Work out the finished part from the listing and answer in its coordinate system (mm). Face numbers are marked on the shaded views. Round coordinates to 2 decimals unless told otherwise and drop trailing zeros. Loops run counter-clockwise (first coordinate to the right, second up) from the corner with the lowest first, then second, coordinate; pieces in that order, holes last. Notation, with made-up numbers: M 1.5,3 L 17.5,3 A32 ccw 17.5,41 Z; hole C 18.5,32.5 d1. An arc over 180 degrees is marked long. One line per item, written item: value.
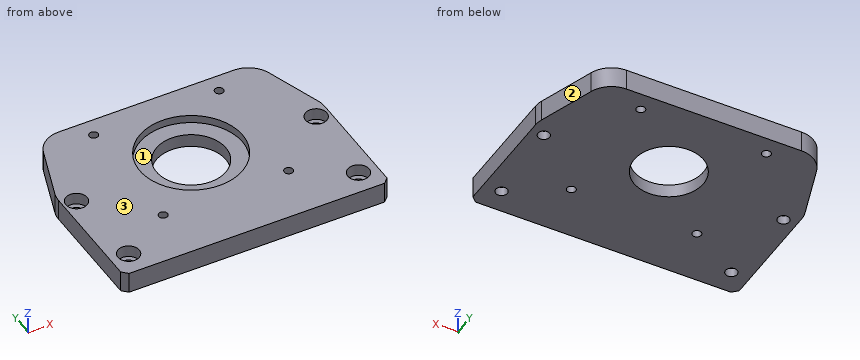
```python
from build123d import *

# Parameters (mm, degrees)
SKETCH_1_W                = 100
SKETCH_1_H                = 75
EXTRUDE_1_DEPTH           = 8
CUT_EXTRUDE_1_DEPTH       = 10
FILLET_1_R                = 10
CHAMFER_2_SIZE            = 2
SKETCH_6_R                = 19.25
CUT_EXTRUDE_2_DEPTH       = 3
SKETCH_7_R                = 13
CUT_EXTRUDE_3_DEPTH       = 63.69968102
HOLE_WIZARD_1_D           = 4.4
HOLE_WIZARD_1_CBORE_D     = 8
HOLE_WIZARD_1_CBORE_DEPTH = 4.5
HOLE_WIZARD_M4_1_D        = 3.3


with BuildPart() as part:
    # 草图1 → 凸台-拉伸1 (new body)
    with BuildSketch(Plane.XY):
        Rectangle(SKETCH_1_W, SKETCH_1_H)
    extrude(amount=EXTRUDE_1_DEPTH)

    # 草图3 → 切除-拉伸1 (cut)
    with BuildSketch(Plane(origin=(0, 0, 0), x_dir=(-1, 0, 0), z_dir=(0, 0, -1))):
        Polygon((-50, 8.5), (-40, 37.5), (-50, 37.5), align=None)
        Polygon((50, 37.5), (50, 8.5), (40, 37.5), align=None)
    extrude(amount=-CUT_EXTRUDE_1_DEPTH, mode=Mode.SUBTRACT)

    # 圆角1
    fillet_1_edges = [part.edges().sort_by_distance(p)[0] for p in [
        (50, 8.5, 4),
        (40, 37.5, 4),
        (-40, 37.5, 4),
        (-50, 8.5, 4),
    ]]
    fillet(fillet_1_edges, radius=FILLET_1_R)

    # 倒角2
    chamfer_2_edges = [part.edges().sort_by_distance(p)[0] for p in [
        (50, -37.5, 4),
        (-50, -37.5, 4),
    ]]
    chamfer(chamfer_2_edges, length=CHAMFER_2_SIZE)

    # 草图6 → 切除-拉伸2 (cut)
    with BuildSketch(Plane.XY.offset(8)):
        with Locations((0, 7)):
            Circle(SKETCH_6_R)
    extrude(amount=-CUT_EXTRUDE_2_DEPTH, mode=Mode.SUBTRACT)

    # 草图7 → 切除-拉伸3 (cut, through all)
    with BuildSketch(Plane.XY.offset(5)):
        with Locations((0, 7)):
            Circle(SKETCH_7_R)
    extrude(amount=-CUT_EXTRUDE_3_DEPTH, mode=Mode.SUBTRACT)

    # 打孔尺寸(%根据)内六角圆柱头螺钉的类型1 (through all)
    with Locations(Plane.XY.offset(8)):
        with Locations((-45, 3.5), (-43.15, -28.5), (43.15, -28.5), (45, 3.5)):
            CounterBoreHole(HOLE_WIZARD_1_D / 2, HOLE_WIZARD_1_CBORE_D / 2, HOLE_WIZARD_1_CBORE_DEPTH)

    # M4 螺纹孔1 (through all)
    with Locations(Plane.XY.offset(8)):
        with Locations((-23.57, -16.57), (23.57, -16.57), (23.57, 30.57), (-23.57, 30.57)):
            Hole(HOLE_WIZARD_M4_1_D / 2)


solid = part.part
```
1) Each of these flat-tipped pins is pushed along its axis until it touches: pin 1 (2 mm diameter, centred on x = 15, y = -2, fed in from +Z); pin 2 (21 mm diameter, centred on x = 0, y = 7, fed in from +Z); pin 3 (5.5 mm diameter, centred on x = 23.57, y = 30.57, fed in from -Z); pin 4 (6.5 mm diameter, centred on x = 43.15, y = -28.5, fed in from +Z). Where does it stop, or does it pass through?
Check values:
pin 1: z = 5
pin 2: through
pin 3: z = 0
pin 4: z = 3.5
2) The mould has two halves that part along X. Classify the marked faces 1, 2 and 3: +X half, -X half, draft (parallel to the pull), parting line (faces both ways), or undercut.
Check values:
face 1: undercut
face 2: +X half
face 3: draft
3) Find section D-D (x = -23.57). Give the vertices of the cut face in (y, z).
Check values:
outline: M -37.5,0 L -18.22,0 L -18.22,8 L -37.5,8 Z; M -14.92,0 L 28.92,0 L 28.92,8 L -14.92,8 Z; M 32.22,0 L 37.5,0 L 37.5,8 L 32.22,8 Z
4) Find the intervals of material crossed by probe 1 along Y at (x, z) = (-23.57, 4); probe 2 along X at (y, z) = (-28, 4.5); probe 3 along Y at (x, z) = (0, 5.7), in increasing order. Write a range as from..to.
Check values:
probe 1: -37.5..-18.22, -14.92..28.92, 32.22..37.5
probe 2: -50..-47.12, -39.18..39.18, 47.12..50
probe 3: -37.5..-12.25, 26.25..37.5
5) Find section A-A (z = 1.25). Give the number of separate pieces and of enclosed holes in the cut face, then the cut area to 3 significant figures.
Check values:
separate pieces: 1
enclosed holes: 9
area: 6,560 mm2
6) Find section B-B (y = -16.57). Give the vertices of the cut face in (x, z), then the cut area to 3 significant figures.
Check values:
outline: M -50,0 L -25.22,0 L -25.22,8 L -50,8 Z; M -21.92,0 L 21.92,0 L 21.92,8 L -21.92,8 Z; M 25.22,0 L 50,0 L 50,8 L 25.22,8 Z
area: 747 mm2
7) Find section C-C (x = 0). Give the vertices of the cut face in (y, z).
Check values:
outline: M -37.5,0 L -6,0 L -6,5 L -12.25,5 L -12.25,8 L -37.5,8 Z; M 20,0 L 37.5,0 L 37.5,8 L 26.25,8 L 26.25,5 L 20,5 Z
